For this review, use the dimensioned drawing (mm, ordinates from the lowest corner) and the shaded views. A direction names the side the tool comes from. Coordinates: 2 decimals unless noted, no trailing zeros. Loops run counter-clockwise (first coordinate to the right, second up) from the corner with the lowest first, then second, coordinate; pieces in that order, holes last. Notation, with made-up numbers: M 84.25,-35.5 L 88.25,-35.5 A14 cw 88.25,-8.5 Z; hole C 6.5,79 d6. An arc over 180 degrees is marked long. Use CSV: the item, a comma, the result in double quotes. Start each with the question number.
1. Draft analysis for pull direction X (two halves, no side actions). For the marked faces 4, 5 and 6, state which applies: +X half, -X half, draft (parallel to the pull), parting line (faces both ways), or undercut.
2. Add section B-B, the plane x = 67.5. Write out the cut boundary in (y, z).
3. For L1, parallel to Z at x = 75, y = 32; L2, parallel to Z at x = 18, y = 23.5; L3, parallel to X at y = 25, z = 25, list the stretches that pass through material, from the lowest coordinate up.
4. Tool access review of the marked faces 1, 2 and 3: name each direction out of +Z, -Z, +X, -X, +Y, -Y from which nothing blocks a thin tool from reaching the whole face with its end or side.
5. Add section C-C, the plane y = 29. Write out the cut boundary in (x, z).
6. Add section D-D, the plane x = 36. Write out the cut boundary in (y, z).
7. Add section A-A, the plane z = 25. Write out the cut boundary in (x, y), then the cut area to 3 significant figures.
8. Clearance check with flat-ended pins moving along their axes: P1, Ø5, axis at x = 29.5, z = 12.5, coming from the -Y side; P2, Ø12, axis at y = 8.5, z = 23, coming from the -X side; P3, Ø9, axis at x = 3, y = 24, coming from the -Z side; P4, Ø16, axis at x = 18, z = 25, coming from the -Y side. State where each tip first meets the part, or that it passes through.
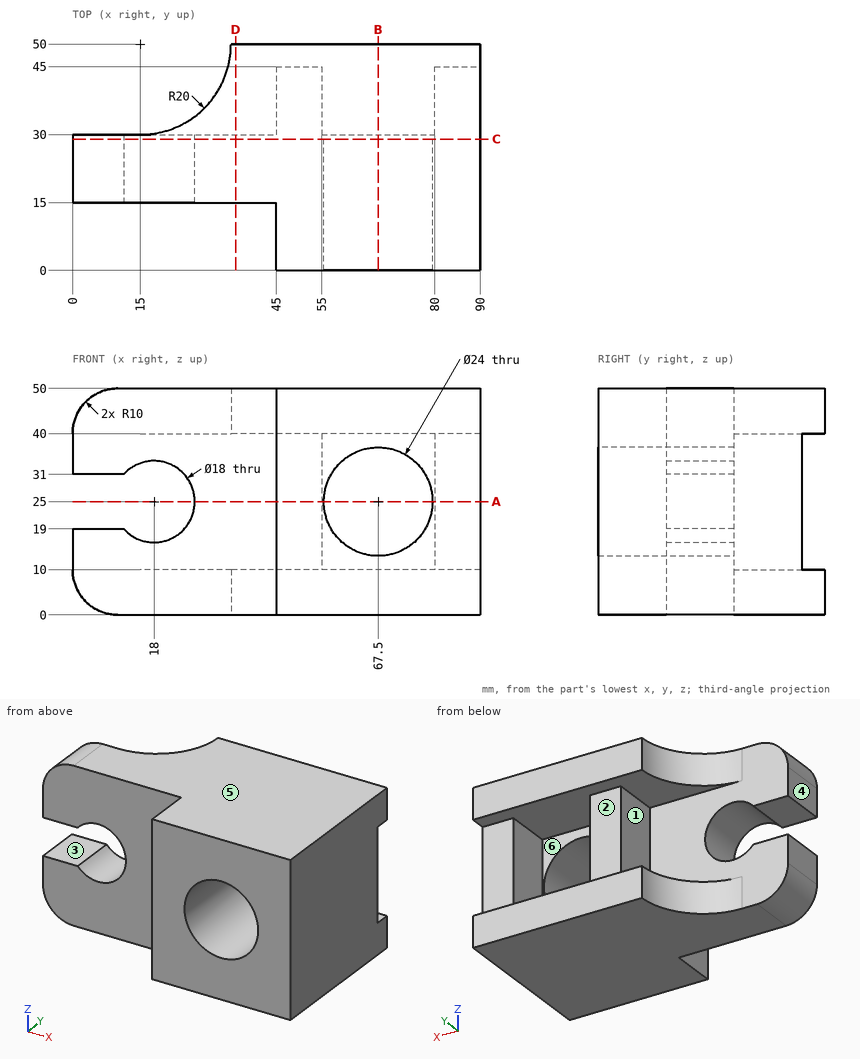
Computed:
1,face 4,"-X half"
1,face 5,"draft"
1,face 6,"undercut"
2,outline,"M 0,0 L 50,0 L 50,10 L 30,10 L 30,13 L 0,13 Z; M 0,37 L 30,37 L 30,40 L 50,40 L 50,50 L 0,50 Z"
3,L1,"z = 0 to 10, 40 to 50"
3,L2,"z = 0 to 16, 34 to 50"
3,L3,"x = 27 to 55.5, 79.5 to 90"
4,face 1,"-X, +Y"
4,face 2,"+X, -X, +Y"
4,face 3,"-X, +Y, -Y"
5,outline,"M 0,10 A10 ccw 10,0 L 90,0 L 90,50 L 10,50 A10 ccw 0,40 L 0,31 L 11.29,31 A9 cw long 11.29,19 L 0,19 Z; hole C 67.5,25 d24"
6,outline,"M 15,0 L 50,0 L 50,10 L 30,10 L 30,40 L 50,40 L 50,50 L 15,50 Z"
7,outline,"M 27,15 L 45,15 L 45,0 L 55.5,0 L 55.5,30 L 55,30 L 55,45 L 45,45 L 45,30 L 27,30 Z; M 79.5,0 L 90,0 L 90,45 L 80,45 L 80,30 L 79.5,30 Z"
7,area,"1,200 mm^2"
8,P1,"stops at y = 15"
8,P2,"stops at x = 45"
8,P3,"stops at z = 0.32"
8,P4,"passes through"
